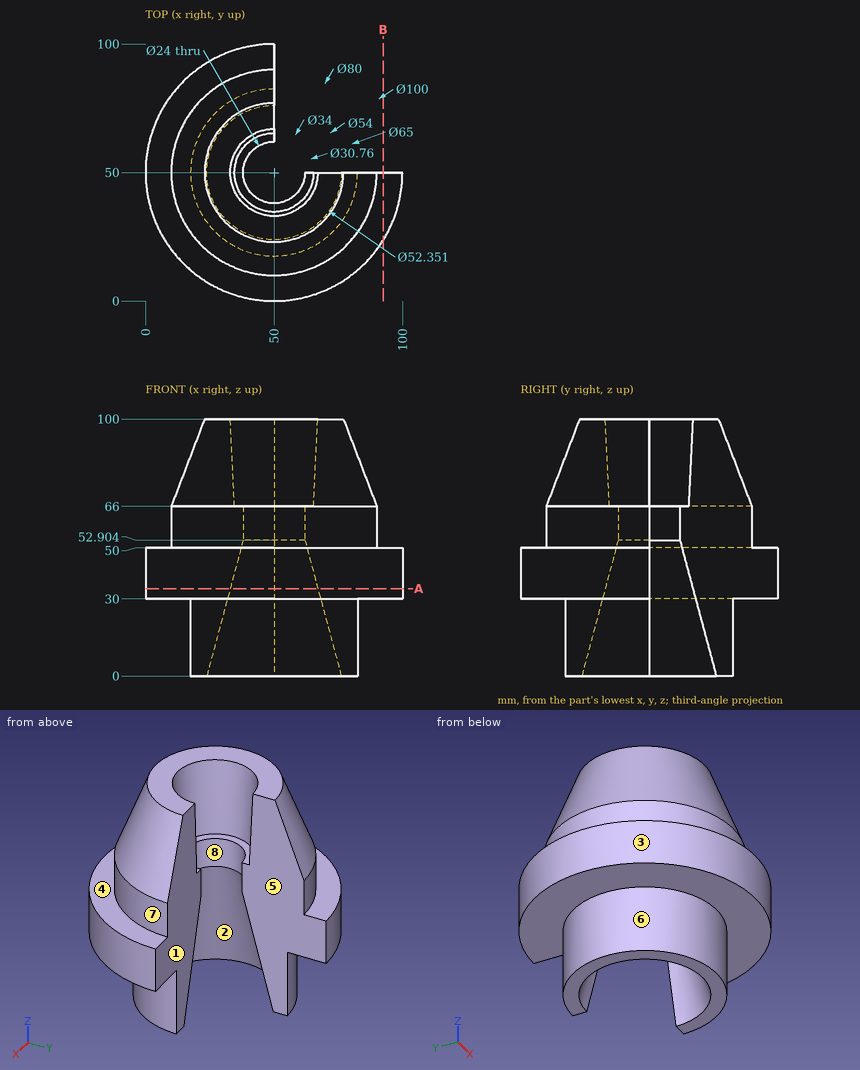
Here's the drawing with two shaded views (mm, measured from the low corner). I have some questions. A direction names the side the tool comes from. Give positions to 0.01 mm unless a question says otherwise; leave off trailing zeros. Order: outer loops, then holes, each group sorted by start corner. A loop starts at its lowest first (then second) coordinate and runs counter-clockwise, first axis right, second up. Notation, with made-up numbers: (10.5, 41.5) - (46.5, 41.5) arc R22 cw to (46.5, 58.5) - close; hole circle Ø1 at (61, 60.5). An arc over 180 degrees is marked (long way). Use a Markdown table: item, result. Add a question column.
Q1. Please list where these lines run through material, in increasing order: line 1 along Y through (x, z) = (33, 28) (1 decimal); line 2 along Z through (x, y) = (8.5, 56.5); line 3 along X through (y, z) = (39.5, 20) (1 decimal).
Q2. If we mould it in two halves opening along Y, with no side actions, what happens to the marked faces 1, 2, 3 and 4? For each: released by +Y, released by -Y, zero draft, split by the parting line, or undercut.
Q3. If we section it at B-B on x = 92.5: Write out the boundary of the cut face in (y, z).
Q4. If we section it at A-A on z = 34: Write out the boundary of the cut face in (x, y) (1 decimal).
Q5. On a 3-axis mill with a long thin cutter (end or side, diameter ignored), from which of +Z, -Z, +X, -X, +Y, -Y can I reach the whole of each face in a straight line? I mean the marked faces 5, 6, 7 and 8. Say none if no direction works.
Q6. I'm going to push flat-ended pins straight in: pin 1 (1 mm diameter, centred on y = 85, z = 57.5, fed in from +X); pin 2 (10 mm diameter, centred on x = 62, z = 89.5, fed in from +Y); pin 3 (5 mm diameter, centred on x = 41.5, z = 10.5, fed in from +Y). Where does each tip first touch, or does it pass through?
Answers follow:
| question | item | result |
|---|---|---|
| 1 | line 1 | y = 22.3 to 42.3, 57.7 to 77.7 |
| 1 | line 2 | z = 30 to 50 |
| 1 | line 3 | x = 19.2 to 32, 68 to 80.8 |
| 2 | face 1 | released by +Y |
| 2 | face 2 | undercut |
| 2 | face 3 | split by the parting line |
| 2 | face 4 | zero draft |
| 3 | outline | (23.66, 30) - (50, 30) - (50, 50) - (23.66, 50) - close |
| 4 | outline | (50, 67.1) - (50, 100) arc R50 ccw (long way) to (100, 50) - (67.1, 50) arc R17.1 cw (long way) to start |
| 5 | face 5 | +Z, -Z, +X, +Y |
| 5 | face 6 | -Z |
| 5 | face 7 | +Z |
| 5 | face 8 | +Z, -Z |
| 6 | pin 1 | stops at x = 50 |
| 6 | pin 2 | stops at y = 50 |
| 6 | pin 3 | stops at y = 81.94 |
